The listing builds one solid part. Answer for the finished solid, in the listing's coordinates (mm). Face numbers are marked on the shaded views. A direction names the side the tool comes from. Round coordinates to 2 decimals unless told otherwise and drop trailing zeros. Order: outer loops, then holes, each group sorted by start corner. A loop starts at its lowest first (then second) coordinate and runs counter-clockwise, first axis right, second up. Notation, with made-up numbers: (-19, 20) -> (-7, 20) arc R19 ccw to (-7, 48) -> close; hole circle Ø9 at (85, 68). An arc over 180 degrees is marked (long way). Return JSON: item names as keys, results as strings. Group by question number.
(1) Which of the six approach directions +Z, -Z, +X, -X, +Y, -Y give full straight-line access (tool end or side, diameter ignored) to the marked faces 4 and 5?
(2) The part is cut by section B-B (x = 79). Determine the outline of the cut face in (y, z), plus the area to 3 significant figures.
(3) The part is cut by section A-A (z = 18). Determine the outline of the cut face in (x, y), plus the area to 3 significant figures.
(4) Determine the mould class of the marked faces 1, 2 and 3 for opening direction Y: +Y half, -Y half, draft (parallel to the pull), parting line (faces both ways), or undercut.
(5) The part is cut by section C-C (y = 106.5). Determine the outline of the cut face in (x, z).
(6) Consider line 1 (Y direction, x = -28, z = 65); line 2 (Z direction, x = 68, y = 8). Determine where each line is inside the solid, lowest interval first. Write a range as [from, to].
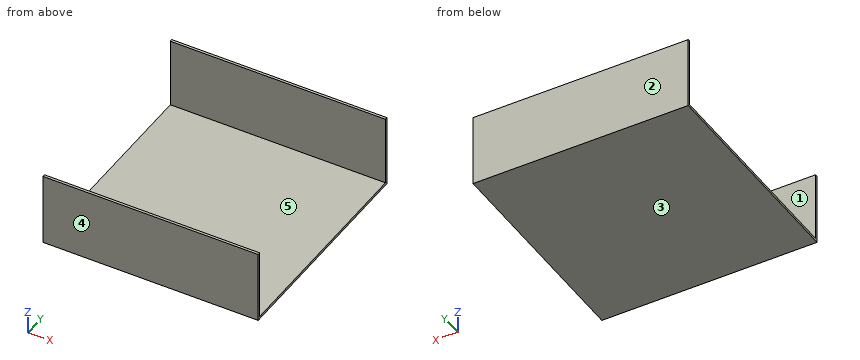
from build123d import *

# Parameters (mm, degrees)
SKETCH1_W           = 246
SKETCH1_H           = 252
BOSS_EXTRUDE1_DEPTH = 3
SKETCH2_W           = 246
SKETCH2_H           = 3
BOSS_EXTRUDE2_DEPTH = 80


with BuildPart() as part:
    # Sketch1 → Boss-Extrude1 (new body)
    with BuildSketch(Plane.XY):
        Rectangle(SKETCH1_W, SKETCH1_H)
    extrude(amount=BOSS_EXTRUDE1_DEPTH)

    # Sketch2 → Boss-Extrude2 (add)
    with BuildSketch(Plane.XY.offset(3)):
        with Locations((0, 124.5)):
            Rectangle(SKETCH2_W, SKETCH2_H)
        with Locations((0, -124.5)):
            Rectangle(SKETCH2_W, SKETCH2_H)
    extrude(amount=BOSS_EXTRUDE2_DEPTH)


solid = part.part
Answer below:
{
 "1": {"face 4": "+Z, -Z, +X, -X, -Y", "face 5": "+Z, +X, -X"},
 "2": {"outline": "(-126, 0) -> (126, 0) -> (126, 83) -> (123, 83) -> (123, 3) -> (-123, 3) -> (-123, 83) -> (-126, 83) -> close", "area": "1,240 mm²"},
 "3": {"outline": "(-123, -126) -> (123, -126) -> (123, -123) -> (-123, -123) -> close; (-123, 123) -> (123, 123) -> (123, 126) -> (-123, 126) -> close", "area": "1,480 mm²"},
 "4": {"face 1": "undercut", "face 2": "+Y half", "face 3": "draft"},
 "5": {"outline": "(-123, 0) -> (123, 0) -> (123, 3) -> (-123, 3) -> close"},
 "6": {"line 1": "y = [-126, -123], [123, 126]", "line 2": "z = [0, 3]"}
}
